Check sheet for the modelled part. Datum: model origin and axes. Units: mm. A direction names the side the tool comes from. Give positions to 0.01 mm unless a question says otherwise; leave off trailing zeros. Order: outer loops, then holes, each group sorted by start corner. A loop starts at its lowest first (then second) coordinate and runs counter-clockwise, first axis right, second up.
Item 1: Gauge pin test, flat ends, axial feed: P1, Ø10, axis at y = 25, z = -11, coming from the +X side; P2, Ø3, axis at x = -11, y = 28.5, coming from the +Z side; P3, Ø4, axis at x = -12.5, y = 10, coming from the +Z side. Record the tip position at first contact, or that the pin passes through.
Item 2: Sectioned sample at C-C on y = 7.5. Record the boundary of the cut face in (x, z), and give its area (3 significant figures).
Item 3: Release check for a two-part mould opening along Y. For faces 1 (the cylindrical face through (-0.325, 10.536, -15.437)), 2 (the flat face through (0, 10, 3)), 3 (the cylindrical face through (-3.755, 4.781, 11.923)), 4 (the cylindrical face through (-0.325, 10.536, 15.481)) record: released by +Y, released by -Y, zero draft, split by the parting line, or undercut.
Item 4: Sectioned sample at A-A on y = 26. Record the boundary of the cut face in (x, z).
Item 5: Access from +Z, -Z, +X, -X, +Y, -Y to the whole of each face (thin tool, end or side, straight path). Record for faces 5 (the flat face through (0, 0, 0)), 6 (the cylindrical face through (5.362, 20.846, 12.932)), 7 (the flat face through (8, 7, 10)).
Item 6: Material ranges on line 1 along X through (y, z) = (25, 0); line 2 along Y through (x, z) = (-11, -8); line 3 along Y through (x, z) = (3, 2.5), recorded low to high.
from build123d import *

# Parameters (mm, degrees)
M6_TAPPED_HOLE1_D     = 5
M6_TAPPED_HOLE1_DEPTH = 5
M6_TAPPED_HOLE1_TIP   = 1.502151548
SKETCH4_R             = 1.5
CUT_EXTRUDE1_DEPTH    = 35


with BuildPart() as part:
    # Sketch1 → Revolve1 (revolve)
    with BuildSketch(Plane.XY, mode=Mode.PRIVATE) as revolve1_sk:
        Polygon((0, 0), (-10, 0), (-12.5, 2.5), (-12.5, 7), (-16, 7), (-17, 8), (-17, 32), (-14, 32), (-14, 10), (0, 10), align=None)
    revolve(revolve1_sk.sketch.rotate(Axis((0, 19.380505724, 0), (0, -1, 0)), 270), axis=Axis((0, 19.380505724, 0), (0, -1, 0)))

    # M6 Tapped Hole1
    with Locations(Plane(origin=(0, 10, 0), x_dir=(1, 0, 0), z_dir=(0, 1, 0))):
        with Locations((0, 0)):
            Hole(M6_TAPPED_HOLE1_D / 2, depth=M6_TAPPED_HOLE1_DEPTH)
            with Locations((0, 0, -(M6_TAPPED_HOLE1_DEPTH + M6_TAPPED_HOLE1_TIP / 2))):  # 118° drill point
                Cone(0, M6_TAPPED_HOLE1_D / 2, M6_TAPPED_HOLE1_TIP, mode=Mode.SUBTRACT)

    # Sketch4 → Cut-Extrude1 (cut, symmetric)
    with BuildSketch(Plane.XY):
        with Locations((0, 12)):
            Circle(SKETCH4_R)
    extrude(amount=CUT_EXTRUDE1_DEPTH, both=True, mode=Mode.SUBTRACT)


solid = part.part
Report:
1. P1: stops at x = 15.91
1. P2: stops at z = 14.1
1. P3: stops at z = 13.37
2. outline: circle Ø33 at (0, 0); hole circle Ø5 at (0, 0)
2. area: 836 mm2
3. face 1: undercut
3. face 2: released by +Y
3. face 3: zero draft
3. face 4: undercut
4. outline: circle Ø34 at (0, 0); hole circle Ø28 at (0, 0)
5. face 5: +Z, -Z, +X, -X, -Y
5. face 6: +Y
5. face 7: -Y
6. line 1: x = -17 to -14, 14 to 17
6. line 2: y = 7 to 10
6. line 3: y = 0 to 10
